Part model, mm, in its own coordinate system. Face numbers are marked on the shaded views. Round coordinates to 2 decimals unless told otherwise and drop trailing zeros. Order: outer loops, then holes, each group sorted by start corner. A loop starts at its lowest first (then second) coordinate and runs counter-clockwise, first axis right, second up. Notation, with made-up numbers: (-13.5, 43) -> (27.5, 43) arc R21 cw to (27.5, 64) -> close; hole circle Ø6 at (89, -35). An arc over 180 degrees is marked (long way). Use CSV: the item, a comma, the result in double quotes.
```python
from build123d import *

# Parameters (mm, degrees)
SKETCH1_R           = 6.499999992
BOSS_EXTRUDE1_DEPTH = 6


with BuildPart() as part:
    # Sketch1 → Boss-Extrude1 (new, symmetric)
    with BuildSketch(Plane.XY):
        with BuildLine():
            Line((249.080198754, 296.842221709), (267.033227589, 318.237808321))
            ThreePointArc((267.033227589, 318.237808321), (295.209868645, 320.702944991), (297.675005315, 292.526303935))
            Line((297.675005315, 292.526303935), (278.391377025, 269.544970642))
            ThreePointArc((278.391377025, 269.544970642), (264.088717655, 283.572564272), (249.080198754, 296.842221709))
        make_face()
        with Locations((282.354116452, 305.382056128)):
            Circle(SKETCH1_R, mode=Mode.SUBTRACT)
    extrude(amount=BOSS_EXTRUDE1_DEPTH, both=True)


solid = part.part
```
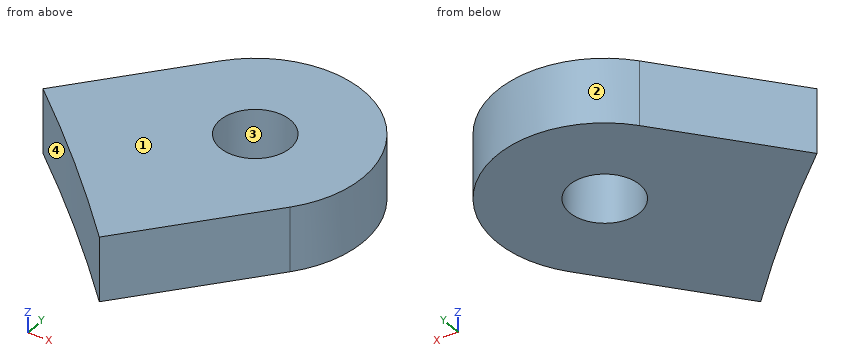
(1) Pull direction X, two halves, no side cores. Call the marked faces 1, 2, 3 and 4: released by +X, released by -X, zero draft, split by the parting line, or undercut.
Reply:
face 1,"zero draft"
face 2,"split by the parting line"
face 3,"undercut"
face 4,"released by -X"
(2) Probe probe 1 along Y at (x, z) = (286.5, -1.75); probe 2 along X at (y, z) = (302, -0.5); probe 3 along Y at (x, z) = (269.5, 4). List the from-to ranges inside material, lowest first. Write a range as [from, to].
Reply:
probe 1,"[279.21, 300.38], [310.39, 324.95]"
probe 2,"[253.41, 276.8], [287.9, 302.07]"
probe 3,"[278.43, 320.7]"
(3) Cut at B-B, the plane z = -2.5. Give the cut face in (x, y) (3 decimals), then the cut area to 3 significant figures.
Reply:
outline,"(249.08, 296.842) arc R387.5 cw to (278.391, 269.545) -> (297.675, 292.526) arc R20 ccw to (267.033, 318.238) -> close; hole circle Ø13 at (282.354, 305.382)"
area,"1,640 mm2"
(4) Cut at C-C, the plane y = 319. Give the cut face in (x, z).
Reply:
outline,"(267.71, -6) -> (297, -6) -> (297, 6) -> (267.71, 6) -> close"
(5) Drop flat-ended pins along their axis: P1, Ø6, axis at y = 286, z = -4, coming from the +X side; P2, Ø2, axis at x = 289, z = 0, coming from the -Y side; P3, Ø3, axis at x = 288.5, z = 1.5, coming from the +Y side. Give the stop position or say it passes through.
Reply:
P1,"x = 294.72"
P2,"y = 281"
P3,"y = 324.83"
(6) Cut at D-D, the plane x = 292. Give the cut face in (y, z).
Reply:
outline,"(285.76, -6) -> (322.9, -6) -> (322.9, 6) -> (285.76, 6) -> close"
(7) Cut at A-A, the plane x = 286. Give the cut face in (y, z), then the cut area to 3 significant figures.
Reply:
outline,"(278.61, -6) -> (300, -6) -> (300, 6) -> (278.61, 6) -> close; (310.76, -6) -> (325.05, -6) -> (325.05, 6) -> (310.76, 6) -> close"
area,"428 mm2"
